Model file for the job. Use its own axes, mm. Give positions to 0.01 mm unless a question says otherwise; leave off trailing zeros. Order: outer loops, then holes, each group sorted by start corner. A loop starts at its lowest first (then second) coordinate and runs counter-clockwise, first axis right, second up. Notation, with made-up numbers: (33, 32) -> (74, 32) arc R26 ccw to (74, 53) -> close; hole circle Ø4 at (52.5, 49). An arc over 180 degrees is marked (long way). Answer in a Markdown table with one row per item. Add a question column.
from build123d import *

# Parameters (mm, degrees)
SKETCH_1_W                       = 538.2
SKETCH_1_H                       = 238
EXTRUDE_1_DEPTH                  = 1.5
HOLE_WIZARD_7_1_7_1_1_AT_2_COUNT = 2
HOLE_WIZARD_7_1_7_1_1_AT_2_PITCH = 216
HOLE_WIZARD_7_1_7_1_1_AT_3_COUNT = 2
HOLE_WIZARD_7_1_7_1_1_AT_3_PITCH = 516.2
FILLET_1_R                       = 3
SKETCH_6_W                       = 35
SKETCH_6_H                       = 75
CUT_EXTRUDE_1_DEPTH              = 1.5
SKETCH_7_R                       = 3.2
CUT_EXTRUDE_2_DEPTH              = 1.5


with BuildPart() as part:
    # 草图1 → 凸台-拉伸1 (new body)
    with BuildSketch(Plane.XY):
        with Locations((36.480246914, 139.567901235)):
            Rectangle(SKETCH_1_W, SKETCH_1_H)
    extrude(amount=-EXTRUDE_1_DEPTH)

    # 草图2 → 孔1 (revolve, cut)
    with BuildSketch(Plane(origin=(-221.619753086, 31.567901235, 0), x_dir=(0, -1, 0), z_dir=(1, 0, 0))):
        Polygon((0, 0), (0, 1.5), (3.45, 1.5), (4.95, 0), align=None)
    revolve(axis=Axis((-221.619753086, 31.567901235, -110), (0, 0, 1)), mode=Mode.SUBTRACT)

    # 草图4 → Ø7.1 (7.1) 直径孔1 (revolve, cut)
    with BuildSketch(Plane(origin=(294.580246914, 247.567901235, 0), x_dir=(0, -1, 0), z_dir=(1, 0, 0))):
        Polygon((0, 0), (0, 1.5), (3.55, 1.5), (3.55, 1.4), (4.95, 0), align=None)
    hole_wizard_7_1_7_1_1 = revolve(axis=Axis((294.580246914, 247.567901235, 6.35), (0, 0, -1)), mode=Mode.SUBTRACT)

    # Ø7.1 (7.1) 直径孔1 at 2: Ø7.1 (7.1) 直径孔1 ×2
    with Locations(*[(0, -i * HOLE_WIZARD_7_1_7_1_1_AT_2_PITCH, 0) for i in range(1, HOLE_WIZARD_7_1_7_1_1_AT_2_COUNT)]):
        add(hole_wizard_7_1_7_1_1, mode=Mode.SUBTRACT)

    # Ø7.1 (7.1) 直径孔1 at 3: Ø7.1 (7.1) 直径孔1 ×2
    with Locations(*[(-i * HOLE_WIZARD_7_1_7_1_1_AT_3_PITCH, 0, 0) for i in range(1, HOLE_WIZARD_7_1_7_1_1_AT_3_COUNT)]):
        add(hole_wizard_7_1_7_1_1, mode=Mode.SUBTRACT)

    # 圆角1
    fillet_1_edges = [part.edges().sort_by_distance(p)[0] for p in [
        (-232.619753086, 258.567901235, -0.75),
        (305.580246914, 258.567901235, -0.75),
        (305.580246914, 20.567901235, -0.75),
        (-232.619753086, 20.567901235, -0.75),
    ]]
    fillet(fillet_1_edges, radius=FILLET_1_R)

    # 草图6 → 切除-拉伸1 (cut)
    with BuildSketch(Plane.XY):
        with Locations((-9.919753086, 139.567901235)):
            Rectangle(SKETCH_6_W, SKETCH_6_H)
    extrude(amount=-CUT_EXTRUDE_1_DEPTH, mode=Mode.SUBTRACT)

    # 草图7 → 切除-拉伸2 (cut)
    with BuildSketch(Plane.XY):
        with Locations((2.580246914, 94.067901235)):
            Circle(SKETCH_7_R)
        with Locations((-22.419753086, 94.067901235)):
            Circle(SKETCH_7_R)
        with Locations((2.580246914, 185.067901235)):
            Circle(SKETCH_7_R)
        with Locations((-22.419753086, 185.067901235)):
            Circle(SKETCH_7_R)
    extrude(amount=-CUT_EXTRUDE_2_DEPTH, mode=Mode.SUBTRACT)


solid = part.part
Item 1: Saw through at A-A on y = 113. List the corners of the cut face in (x, z).
Item 2: Saw through at B-B on z = -1. Give the number of separate pieces and of enclosed holes in the cut face, plus the area to 3 significant figures.
Item 3: Pin check, flat tip, straight feed: pin 1 Ø10 at (x, y) = (-22.42, 185.07) entering from +Z. Stop position of the tip, or through.
Item 4: Wall check: line 1 (Y direction, x = -3.5, z = -1.1); line 2 (X direction, y = 130, z = -0.1). Give the ranges that are in metal, low to high.
Evaluation:
| question | item | result |
|---|---|---|
| 1 | outline | (-232.62, -1.5) -> (-27.42, -1.5) -> (-27.42, 0) -> (-232.62, 0) -> close; (7.58, -1.5) -> (305.58, -1.5) -> (305.58, 0) -> (7.58, 0) -> close |
| 2 | separate pieces | 1 |
| 2 | enclosed holes | 9 |
| 2 | area | 125,000 mm2 |
| 3 | pin 1 | stops at z = 0 |
| 4 | line 1 | y = 20.57 to 102.07, 177.07 to 258.57 |
| 4 | line 2 | x = -232.62 to -27.42, 7.58 to 305.58 |
